Design review of the part shown in the three views and the two pictorial views. Dimensions are in mm from the part's minimum x, y and z. A direction names the side the tool comes from. Coordinates: 2 decimals unless noted, no trailing zeros. Loops run counter-clockwise (first coordinate to the right, second up) from the corner with the lowest first, then second, coordinate; pieces in that order, holes last. Notation, with made-up numbers: M 49,76.25 L 77,76.25 A12 cw 77,84.25 Z; hole C 83,75.25 d9. An arc over 180 degrees is marked long. Put each result on its own line as item: value. Start each with the question number.
(1) Take a section at A-A, the plane y = 15. Give the boundary of the cut face in (x, z), then the cut area to 3 significant figures.
(2) Take a section at C-C, the plane z = 3.65. Give the boundary of the cut face in (x, y).
(3) For probe 1 along X at (y, z) = (3.25, 4.45); probe 2 along Y at (x, z) = (15, 0.35), list the stretches that pass through material, from the lowest coordinate up. Write a range as [from, to].
(4) The part is to be moulded in two halves that separate along Y. For the marked faces 3, 4 and 5, say which applies: +Y half, -Y half, draft (parallel to the pull), parting line (faces both ways), or undercut.
(5) Clearance check with a flat-ended pin moving along its axis: pin 1 (8.5 mm diameter, centred on x = 9.5, y = 8.5, fed in from +Z). State where the tip first meets the part, or that it passes through.
(6) For the marked faces 1 and 2, list the 3-axis set-ups (+Z, -Z, +X, -X, +Y, -Y) from which the entire face can be reached by the end or side of a thin tool; tool diameter is ignored.
(7) Take a section at D-D, the plane y = 2.5. Give the boundary of the cut face in (x, z).
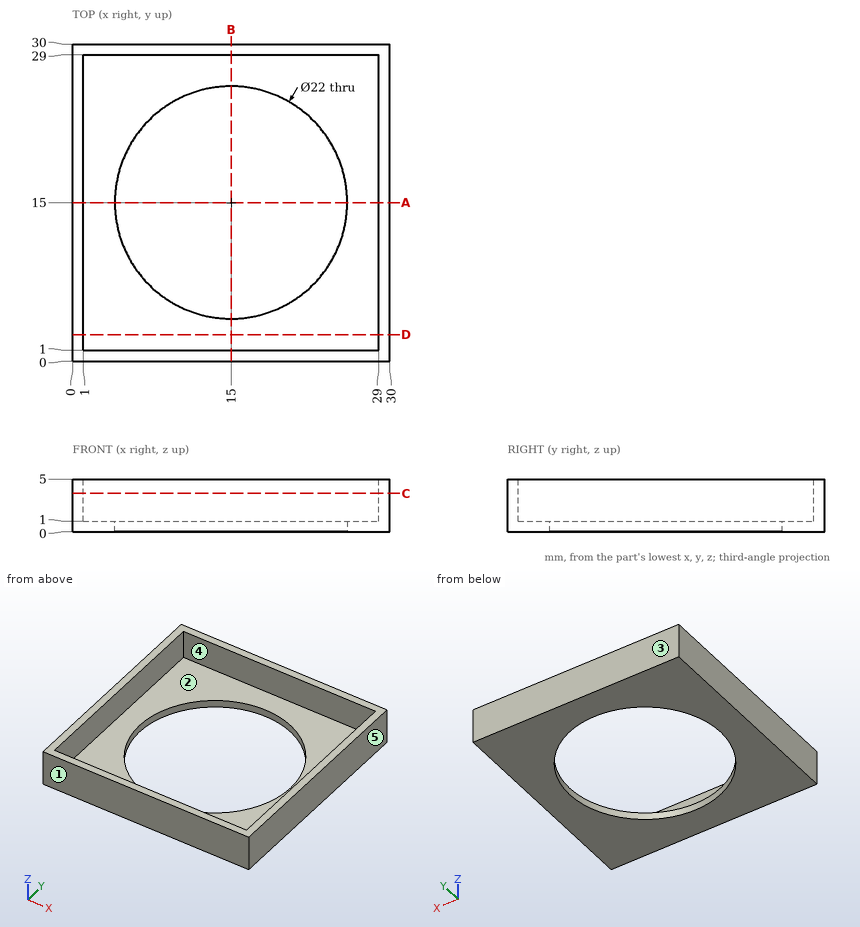
Computed values:
1. outline: M 0,0 L 4,0 L 4,1 L 1,1 L 1,5 L 0,5 Z; M 26,0 L 30,0 L 30,5 L 29,5 L 29,1 L 26,1 Z
1. area: 16.0 mm^2
2. outline: M 0,0 L 30,0 L 30,30 L 0,30 Z; hole M 1,1 L 29,1 L 29,29 L 1,29 Z
3. probe 1: x = [0, 1], [29, 30]
3. probe 2: y = [0, 4], [26, 30]
4. face 3: +Y half
4. face 4: undercut
4. face 5: draft
5. pin 1: stops at z = 1
6. face 1: +Z, -Z, +X, -X, -Y
6. face 2: +Z
7. outline: M 0,0 L 30,0 L 30,5 L 29,5 L 29,1 L 1,1 L 1,5 L 0,5 Z
